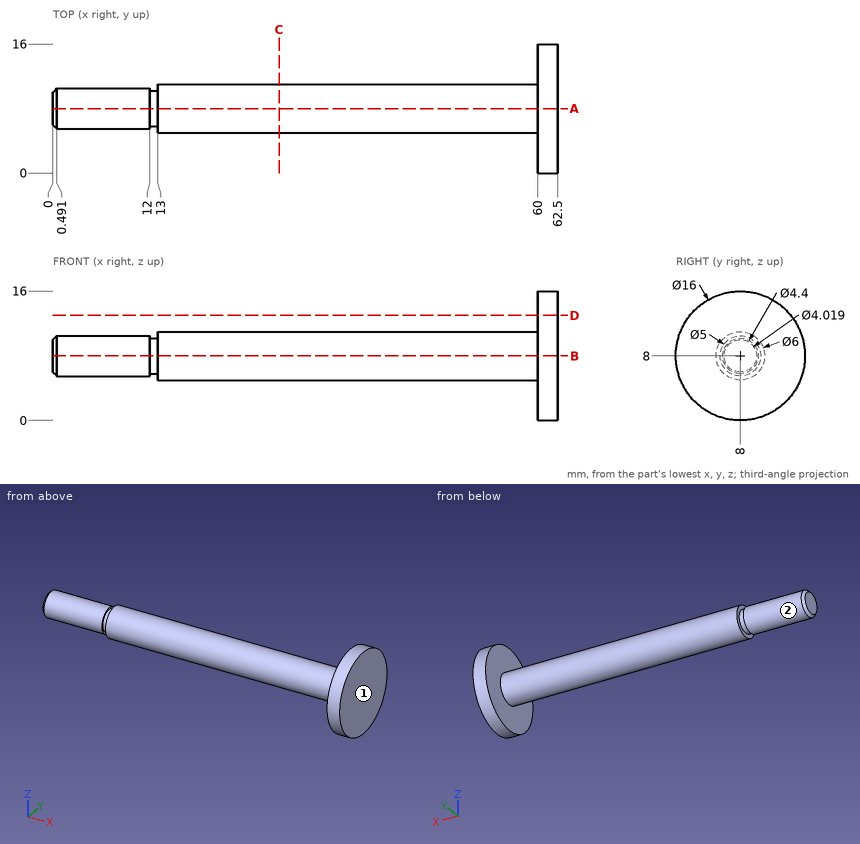
Geometry check sheet. Reference: drawing and pictorial views, mm from the part's lowest x, y, z. A direction names the side the tool comes from. Round coordinates to 2 decimals unless told otherwise and drop trailing zeros. Write each loop counter-clockwise with the first axis right and the second up, starting at its lowest first coordinate (ties: lowest second). Pieces come first, ordered by that corner, then holes.
(1) Section check A-A (y = 8). Enter the section's corners in (x, z), plus the area to 3 significant figures.
Returned:
outline: (0, 5.99) - (0.49, 5.5) - (12, 5.5) - (12, 5.8) - (13, 5.8) - (13, 5) - (60, 5) - (60, 0) - (62.5, 0) - (62.5, 16) - (60, 16) - (60, 11) - (13, 11) - (13, 10.2) - (12, 10.2) - (12, 10.5) - (0.49, 10.5) - (0, 10.01) - close
area: 386 mm2
(2) Section check C-C (x = 28). Enter the section's corners in (y, z).
Returned:
outline: circle Ø6 at (8, 8)
(3) Access from +Z, -Z, +X, -X, +Y, -Y to the whole of each face (thin tool, end or side, straight path). Record for the marked faces 1 and 2.
Returned:
face 1: +Z, -Z, +X, +Y, -Y
face 2: -X
(4) Section check D-D (z = 13). Enter the section's corners in (x, y) (1 decimal).
Returned:
outline: (60, 1.8) - (62.5, 1.8) - (62.5, 14.2) - (60, 14.2) - close
(5) Material ranges on line 1 (X direction, y = 10, z = 4.75); line 2 (Y direction, x = 53, z = 9.75) (1 decimal); line 3 (Z direction, x = 10, y = 7), recorded low to high.
Returned:
line 1: x = 60 to 62.5
line 2: y = 5.6 to 10.4
line 3: z = 5.71 to 10.29
(6) Depth check by flat-ended pin: pin 1 Ø3 at (x, y) = (10, 8.5) entering from -Z; pin 2 Ø3 at (x, z) = (52, 2.5) entering from +Y; pin 3 Ø6 at (y, z) = (14, 13.5) entering from -X; pin 4 Ø1.5 at (x, z) = (44, 8) entering from +Y. Enter the tip coordinate at first touch or a pass-through.
Returned:
pin 1: stops at z = 5.5
pin 2: passes through
pin 3: stops at x = 60
pin 4: stops at y = 11
